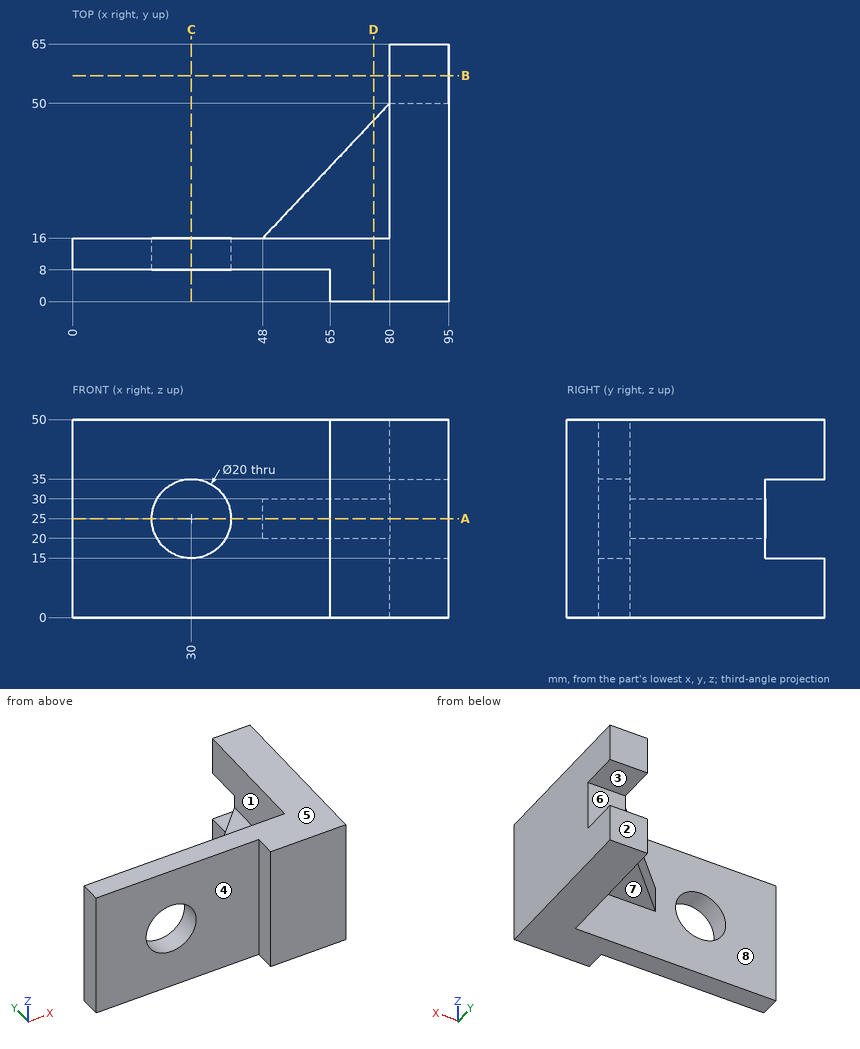
Geometry: see drawing. Coordinates: mm, zero at the bounding-box minimum. A direction names the side the tool comes from. Coordinates: 2 decimals unless noted, no trailing zeros. Write each loop counter-clockwise with the first axis right and the second up, starting at its lowest first coordinate (ties: lowest second). Pieces come first, ordered by that corner, then holes.
1) Section A-A on z = 25. Output: boundary loops of the cut face in (x, y).
2) Pin query (flat end, axial travel): pin 1 Ø15 at (x, z) = (34.5, 35) entering from -Y; pin 2 Ø16 at (x, y) = (60, 40.5) entering from -Z; pin 3 Ø12 at (x, z) = (88.5, 25) entering from +Y; pin 4 Ø1 at (y, z) = (33.5, 27.5) entering from -X. Return the tip coordinate at first contact, or that it passes through.
3) Section C-C on x = 30. Output: boundary loops of the cut face in (y, z).
4) Section D-D on x = 76. Output: boundary loops of the cut face in (y, z), and give its area (3 significant figures).
5) Section B-B on y = 57. Output: boundary loops of the cut face in (x, z), and give its area (3 significant figures).
6) Material intervals for line 1 along Y through (x, z) = (4.5, 8); line 2 along X through (y, z) = (25, 39.5); line 3 along X through (y, z) = (10.5, 25), sorted ascending.
7) Set-up query: the marked faces 1, 2, 3 and 4. Return all of +Z, -Z, +X, -X, +Y, -Y with unobstructed straight access to the full face (end or side cutting, diameter ignored); none if empty.
8) Mould query, pull axis Z, two halves, no side actions, for the marked faces 5, 6, 7 and 8. Classes: pulls with the +Z half, pulls with the -Z half, needs draft (parallel to the pull), parting line crosses it, or undercut.
Check result:
1. outline: (0, 8) - (20, 8) - (20, 16) - (0, 16) - close; (40, 8) - (65, 8) - (65, 0) - (95, 0) - (95, 50) - (80, 50) - (48, 16) - (40, 16) - close
2. pin 1: stops at y = 8
2. pin 2: passes through
2. pin 3: stops at y = 50
2. pin 4: stops at x = 64
3. outline: (8, 0) - (16, 0) - (16, 15) - (8, 15) - close; (8, 35) - (16, 35) - (16, 50) - (8, 50) - close
4. outline: (0, 0) - (16, 0) - (16, 20) - (45.75, 20) - (45.75, 30) - (16, 30) - (16, 50) - (0, 50) - close
4. area: 1,100 mm2
5. outline: (80, 0) - (95, 0) - (95, 15) - (80, 15) - close; (80, 35) - (95, 35) - (95, 50) - (80, 50) - close
5. area: 450 mm2
6. line 1: y = 8 to 16
6. line 2: x = 80 to 95
6. line 3: x = 0 to 20, 40 to 95
7. face 1: +Z, -X, +Y
7. face 2: +Z, -Z, +X, -X, +Y
7. face 3: +X, -X, +Y
7. face 4: +Z, -Z, -X, -Y
8. face 5: pulls with the +Z half
8. face 6: undercut
8. face 7: pulls with the -Z half
8. face 8: needs draft
